Verification items for the finished model (mm, model axes). A direction names the side the tool comes from. Round coordinates to 2 decimals unless told otherwise and drop trailing zeros. Loops run counter-clockwise (first coordinate to the right, second up) from the corner with the lowest first, then second, coordinate; pieces in that order, holes last. Notation, with made-up numbers: (40.25, -9.5) - (79.25, -9.5) arc R14 cw to (79.25, -4.5) - close; hole circle Ø10 at (18.5, 77.25). An arc over 180 degrees is marked (long way). Use CSV: the item, a comma, the result in double quotes.
```python
from build123d import *

# Parameters (mm, degrees)
BASE_PLATE_SKETCH_W              = 85
BASE_PLATE_SKETCH_H              = 140
BASE_PLATE_140X85X18_DEPTH       = 18
UNDERSIDE_RELIEF_GROOVE_SKETCH_W = 49
UNDERSIDE_RELIEF_GROOVE_SKETCH_H = 3
UNDERSIDE_RELIEF_GROOVE_DEPTH    = 150
ANGLED_SUPPORT_WEB_SKETCH_R      = 20
ANGLED_SUPPORT_WEB_SKETCH_R_2    = 9
ANGLED_SUPPORT_WEB_SKETCH_R_3    = 27.5
ANGLED_SUPPORT_WEB_SKETCH_R_4    = 15
ANGLED_SUPPORT_WEB_DEPTH         = 12
UPPER_BOSS_SKETCH_R              = 20
UPPER_BOSS_SKETCH_R_2            = 9
UPPER_BOSS_40_DEPTH              = 12
LOWER_START                      = 12
LOWER_BOSS_SKETCH_A_R            = 27.5
LOWER_BOSS_SKETCH_A_R_2          = 15
LOWER_BOSS_30_A_DEPTH            = 12
LOWER_BOSS_SKETCH_B_R            = 27.5
LOWER_BOSS_SKETCH_B_R_2          = 15
LOWER_BOSS_30_B_DEPTH            = 12
BASE_MOUNTING_HOLES_SKETCH_R     = 8
BASE_MOUNTING_HOLES_2X_16_DEPTH  = 20


with BuildPart() as part:
    # Base Plate Sketch → Base Plate 140x85x18 (new body)
    with BuildSketch(Plane(origin=(0, 0, 0), x_dir=(1, 0, 0), z_dir=(0, 1, 0))):
        Rectangle(BASE_PLATE_SKETCH_W, BASE_PLATE_SKETCH_H)
    extrude(amount=BASE_PLATE_140X85X18_DEPTH)

    # Underside Relief Groove Sketch → Underside Relief Groove (cut)
    with BuildSketch(Plane.XY.offset(70)):
        with Locations((0, 1.5)):
            Rectangle(UNDERSIDE_RELIEF_GROOVE_SKETCH_W, UNDERSIDE_RELIEF_GROOVE_SKETCH_H)
    extrude(amount=-UNDERSIDE_RELIEF_GROOVE_DEPTH, mode=Mode.SUBTRACT)

    # Angled Support Web Sketch → Angled Support Web (add)
    # profile 1 of 3: a face of its own
    with BuildSketch(Plane.ZY.offset(42.5)):
        with BuildLine():
            Line((-70, 18), (70, 18))
            Line((70, 18), (70, 56))
            ThreePointArc((70, 56), (35.857864376, 41.857864376), (50, 76))
            Line((50, 76), (32.5, 76))
            ThreePointArc((32.5, 76), (14.82233047, 83.32233047), (7.5, 101))
            Line((7.5, 101), (7.5, 118))
            ThreePointArc((7.5, 118), (-20, 90.5), (-47.5, 118))
            Line((-47.5, 118), (-70, 18))
        make_face()
    # profile 2 of 3: a face of its own
    with BuildSketch(Plane.ZY.offset(42.5)):
        with Locations((50, 56)):
            Circle(ANGLED_SUPPORT_WEB_SKETCH_R)
        with Locations((50, 56)):
            Circle(ANGLED_SUPPORT_WEB_SKETCH_R_2, mode=Mode.SUBTRACT)
    # profile 3 of 3: a face of its own
    with BuildSketch(Plane.ZY.offset(42.5)):
        with Locations((-20, 118)):
            Circle(ANGLED_SUPPORT_WEB_SKETCH_R_3)
        with Locations((-20, 118)):
            Circle(ANGLED_SUPPORT_WEB_SKETCH_R_4, mode=Mode.SUBTRACT)
    extrude(amount=-ANGLED_SUPPORT_WEB_DEPTH)

    # Upper Boss Sketch → Upper Boss Ø40 (add)
    with BuildSketch(Plane(origin=(-30.5, 0, 0), x_dir=(0, 0, -1), z_dir=(1, 0, 0))):
        with Locations(Location((-50, 56, 0), (0, 0, 180))):
            Circle(UPPER_BOSS_SKETCH_R)
        with Locations(Location((-50, 56, 0), (0, 0, 180))):
            Circle(UPPER_BOSS_SKETCH_R_2, mode=Mode.SUBTRACT)
    extrude(amount=UPPER_BOSS_40_DEPTH)

    # Lower Boss Sketch A → Lower Boss Ø30 A (add)
    with BuildSketch(Plane.ZY.offset(42.5).offset(LOWER_START)):
        with Locations((-20, 118)):
            Circle(LOWER_BOSS_SKETCH_A_R)
        with Locations((-20, 118)):
            Circle(LOWER_BOSS_SKETCH_A_R_2, mode=Mode.SUBTRACT)
    extrude(amount=-LOWER_BOSS_30_A_DEPTH)

    # Lower Boss Sketch B → Lower Boss Ø30 B (add)
    with BuildSketch(Plane(origin=(-30.5, 0, 0), x_dir=(0, 0, -1), z_dir=(1, 0, 0))):
        with Locations(Location((20, 118, 0), (0, 0, 180))):
            Circle(LOWER_BOSS_SKETCH_B_R)
        with Locations(Location((20, 118, 0), (0, 0, 180))):
            Circle(LOWER_BOSS_SKETCH_B_R_2, mode=Mode.SUBTRACT)
    extrude(amount=LOWER_BOSS_30_B_DEPTH)

    # Base Mounting Holes Sketch → Base Mounting Holes 2xØ16 (cut)
    with BuildSketch(Plane(origin=(0, 18, 0), x_dir=(1, 0, 0), z_dir=(0, 1, 0))):
        with Locations(Location((12.5, 35, 0), (0, 0, 270))):
            Circle(BASE_MOUNTING_HOLES_SKETCH_R)
        with Locations(Location((12.5, -35, 0), (0, 0, 270))):
            Circle(BASE_MOUNTING_HOLES_SKETCH_R)
    extrude(amount=-BASE_MOUNTING_HOLES_2X_16_DEPTH, mode=Mode.SUBTRACT)


solid = part.part
```
1) Access from +Z, -Z, +X, -X, +Y, -Y to the whole of each face (thin tool, end or side, straight path). Record for faces 4 (the face through (-37, 76, 41)), 5 (the face through (-34, 0, -1)), 6 (the face through (7.632, 10.605, 28.651)), 7 (the face through (0, 3, 1)), 8 (the face through (-18.5, 130, -8)).
Returned:
face 4,"+Z, +X, -X, +Y"
face 5,"+Z, -Z, +X, -X, -Y"
face 6,"+Y, -Y"
face 7,"+Z, -Z, -Y"
face 8,"+Z, -Z, +X, +Y"
2) Cross-section at D-D, the plane x = -38. Record the cut outline in (y, z), then the cut area to 3 significant figures.
Returned:
outline,"(0, -70) - (18, -70) - (118, -47.5) arc R27.5 ccw to (118, 7.5) - (101, 7.5) arc R25 cw to (76, 32.5) - (76, 50) arc R20 ccw to (56, 70) - (0, 70) - close; hole circle Ø18 at (56, 50); hole circle Ø30 at (118, -20)"
area,"13,000 mm²"
3) Cross-section at B-B, the plane x = 12.5. Record the cut outline in (y, z).
Returned:
outline,"(3, -70) - (18, -70) - (18, -43) - (3, -43) - close; (3, -27) - (18, -27) - (18, 27) - (3, 27) - close; (3, 43) - (18, 43) - (18, 70) - (3, 70) - close"
4) Cross-section at C-C, the plane y = 13.5. Record the cut outline in (x, z), then the cut area to 3 significant figures.
Returned:
outline,"(-42.5, -70) - (42.5, -70) - (42.5, 70) - (-42.5, 70) - close; hole circle Ø16 at (12.5, -35); hole circle Ø16 at (12.5, 35)"
area,"11,500 mm²"
5) Mould release check, pull along X, two halves, no side actions. Record for faces 1 (the face through (7.632, 10.605, -41.349)), 2 (the face through (5, 18, -1)), 3 (the face through (-18.5, 65, 54)): +X half, -X half, draft (parallel to the pull), parting line (faces both ways), or undercut.
Returned:
face 1,"undercut"
face 2,"draft"
face 3,"+X half"
6) Gauge pin test, flat ends, axial feed: pin 1 Ø20.5 at (y, z) = (56, 50) entering from -X; pin 2 Ø16.5 at (y, z) = (105.5, -8) entering from +X; pin 3 Ø6 at (x, y) = (-39.5, 108.5) entering from +Z. Record the tip position at first contact, or that the pin passes through.
Returned:
pin 1,"stops at x = -42.5"
pin 2,"stops at x = -18.5"
pin 3,"stops at z = 7.5"
7) Thickness scan on probe 1 along Y at (x, z) = (-25.5, -20); probe 2 along Y at (x, z) = (-23.25, -20); probe 3 along Z at (x, y) = (-23, 56). Record the ranges inside material, lowest first. Write a range as [from, to].
Returned:
probe 1,"y = [0, 18], [90.5, 103], [133, 145.5]"
probe 2,"y = [3, 18], [90.5, 103], [133, 145.5]"
probe 3,"z = [30, 41], [59, 70]"
8) Cross-section at A-A, the plane z = -20. Record the cut outline in (x, y), then the cut area to 3 significant figures.
Returned:
outline,"(-54.5, 90.5) - (-42.5, 90.5) - (-42.5, 0) - (-24.5, 0) - (-24.5, 3) - (24.5, 3) - (24.5, 0) - (42.5, 0) - (42.5, 18) - (-30.5, 18) - (-30.5, 90.5) - (-18.5, 90.5) - (-18.5, 103) - (-54.5, 103) - close; (-54.5, 133) - (-18.5, 133) - (-18.5, 145.5) - (-54.5, 145.5) - close"
area,"3,150 mm²"
